Here's how the part is built. I have some questions about the finished solid (model axes, mm). Face numbers are marked on the shaded views. A direction names the side the tool comes from. Coordinates: 2 decimals unless noted, no trailing zeros. Loops run counter-clockwise (first coordinate to the right, second up) from the corner with the lowest first, then second, coordinate; pieces in that order, holes last.
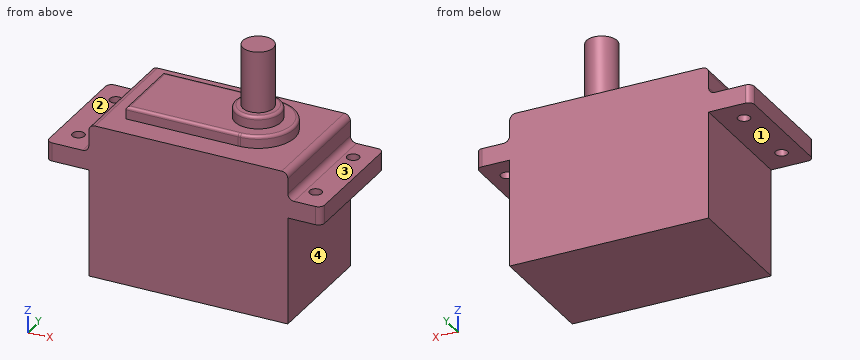
```python
from build123d import *

# Parameters (mm, degrees)
SKETCH1_W           = 65
SKETCH1_H           = 40
BOSS_EXTRUDE1_DEPTH = 50
BOSS_EXTRUDE2_DEPTH = 4
SKETCH3_R           = 7.5
BOSS_EXTRUDE3_DEPTH = 4
SKETCH4_R           = 5
BOSS_EXTRUDE4_DEPTH = 20
FILLET1_R           = 1
SKETCH5_W           = 6
SKETCH5_H           = 40
BOSS_EXTRUDE5_DEPTH = 20
SKETCH6_W           = 6
SKETCH6_H           = 40
BOSS_EXTRUDE6_DEPTH = 20
SKETCH7_R           = 2
SKETCH7_W           = 9
SKETCH7_H           = 40
SKETCH7_W_2         = 6
CUT_EXTRUDE1_DEPTH  = 20
FILLET2_R           = 2
SCALE1_SCALE        = 0.5


with BuildPart() as part:
    # Sketch1 → Boss-Extrude1 (new body)
    with BuildSketch(Plane.XY):
        Rectangle(SKETCH1_W, SKETCH1_H)
    extrude(amount=BOSS_EXTRUDE1_DEPTH)

    # Sketch2 → Boss-Extrude2 (add)
    with BuildSketch(Plane.XY.offset(50)):
        with BuildLine():
            ThreePointArc((12.995819527, -11.993531793), (24.600254242, 0.197000611), (12.601871402, 12))
            Line((12.601871402, 12), (-24.5, 12))
            Line((-24.5, 12), (-24.5, -12.000098614))
            Line((-24.5, -12.000098614), (12.21212427, -11.993669046))
            Line((12.21212427, -11.993669046), (12.995819527, -11.993531793))
        make_face()
    extrude(amount=BOSS_EXTRUDE2_DEPTH)

    # Sketch3 → Boss-Extrude3 (add)
    with BuildSketch(Plane.XY.offset(54)):
        with Locations((12.601871402, 0)):
            Circle(SKETCH3_R)
    extrude(amount=BOSS_EXTRUDE3_DEPTH)

    # Sketch4 → Boss-Extrude4 (add)
    with BuildSketch(Plane.XY.offset(58)):
        with Locations((12.601871402, 0)):
            Circle(SKETCH4_R)
    extrude(amount=BOSS_EXTRUDE4_DEPTH)

    # Fillet1
    fillet1_edges = [part.edges().sort_by_distance(p)[0] for p in [
        (-5.752090236, -11.996815204, 54),
        (24.600254242, 0.197000611, 54),
        (-5.949064299, 12, 54),
        (-24.5, -4.9307e-05, 54),
        (5.101871402, 0, 58),
    ]]
    fillet(fillet1_edges, radius=FILLET1_R)

    # Sketch5 → Boss-Extrude5 (add)
    with BuildSketch(Plane(origin=(32.5, 0, 0), x_dir=(0, 0, -1), z_dir=(1, 0, 0))):
        with Locations((-38, 0)):
            Rectangle(SKETCH5_W, SKETCH5_H)
    extrude(amount=BOSS_EXTRUDE5_DEPTH)

    # Sketch6 → Boss-Extrude6 (add)
    with BuildSketch(Plane.ZY.offset(32.5)):
        with Locations((38, 0)):
            Rectangle(SKETCH6_W, SKETCH6_H)
    extrude(amount=BOSS_EXTRUDE6_DEPTH)

    # Sketch7 → Cut-Extrude1 (cut)
    with BuildSketch(Plane.XY.offset(41)):
        with Locations((-39.98, 12)):
            Circle(SKETCH7_R)
        with Locations((-39.98, -12)):
            Circle(SKETCH7_R)
        with Locations((37.5, 12)):
            Circle(SKETCH7_R)
        with Locations((37.5, -12)):
            Circle(SKETCH7_R)
        with Locations((48, 0)):
            Rectangle(SKETCH7_W, SKETCH7_H)
        with Locations((-49.5, 0)):
            Rectangle(SKETCH7_W_2, SKETCH7_H)
    extrude(amount=-CUT_EXTRUDE1_DEPTH, mode=Mode.SUBTRACT)

    # Fillet2
    fillet2_edges = [part.edges().sort_by_distance(p)[0] for p in [
        (32.5, 0, 50),
        (-46.5, 20, 38),
        (-46.5, -20, 38),
        (-32.5, 0, 50),
        (32.5, 0, 41),
        (-32.5, 0, 41),
        (43.5, -20, 38),
        (43.5, 20, 38),
    ]]
    fillet(fillet2_edges, radius=FILLET2_R)


with BuildPart() as part_1:
    # Scale1: scaled about (0, 0, 0)
    add(part.part.scale(SCALE1_SCALE))


solid = part_1.part
```
1. I want a section at C-C (z = 31). Please give me the cut outline in (x, y), then the cut area to 3 significant figures.
2. I need wall thicknesses on line 1 along X through (y, z) = (-0.5, 7); line 2 along X through (y, z) = (-5.25, 19); line 3 along Z through (x, y) = (0, -4). Which ranges of each line are inside material? Lowest first, please.
3. I want a section at A-A (x = 18.75). Please give me the cut outline in (y, z), then the cut area to 3 significant figures.
4. On a 3-axis mill with a long thin cutter (end or side, diameter ignored), from which of +Z, -Z, +X, -X, +Y, -Y can I reach the whole of each face in a straight line? I mean the marked faces 1, 2, 3 and 4. Say none if no direction works.
5. I want a section at B-B (z = 4.5). Please give me the cut outline in (x, y), then the cut area to 3 significant figures.
6. For pin 1 (2 mm diameter, centred on x = 19, y = -2, fed in from +Z); pin 2 (3 mm diameter, centred on x = 13.5, y = 5.5, fed in from +Z); pin 3 (3 mm diameter, centred on x = 18.75, y = 6, fed in from -Z); pin 4 (6 mm diameter, centred on x = -3.5, y = 3, fed in from -Z), each with a flat end and sliding along its axis, tell me the tip position at first contact or that it passes through.
Response values:
1. outline: circle Ø5 at (6.3, 0)
1. area: 19.6 mm2
2. line 1: x = -16.25 to 16.25
2. line 2: x = -23.25 to -20.65, -19.33 to 18.09, 19.41 to 21.75
2. line 3: z = 0 to 27
3. outline: (-10, 17.5) - (-7, 17.5) - (-7, 20.5) - (-10, 20.5) - close; (-5, 17.5) - (5, 17.5) - (5, 20.5) - (-5, 20.5) - close; (7, 17.5) - (10, 17.5) - (10, 20.5) - (7, 20.5) - close
3. area: 48.0 mm2
4. face 1: -Z, -X, +Y, -Y
4. face 2: +Z, -X, +Y, -Y
4. face 3: +Z, +X, +Y, -Y
4. face 4: -Z, +X, +Y, -Y
5. outline: (-16.25, -10) - (16.25, -10) - (16.25, 10) - (-16.25, 10) - close
5. area: 650 mm2
6. pin 1: stops at z = 20.5
6. pin 2: stops at z = 25
6. pin 3: stops at z = 17.5
6. pin 4: stops at z = 0
